from build123d import *

# Parameters (mm, degrees)
BASE_FLANGE_SKETCH_R = 11
BASE_FLANGE_DEPTH    = 24
HUB_BOSS_SKETCH_72_R = 36
HUB_BOSS_72_DEPTH    = 38
WEDGE_SUPPORT_DEPTH  = 28
BORE_28_REACH        = 176.416
BORE_SKETCH_28_R     = 14


with BuildPart() as part:
    # Base Flange Sketch → Base Flange (new body)
    with BuildSketch(Plane(origin=(0, 0, 0), x_dir=(1, 0, 0), z_dir=(0, 1, 0))):
        with BuildLine():
            Line((-116, 54.332778116), (-60, 54.332778116))
            ThreePointArc((-60, 54.332778116), (-42.391267518, 43.899782505), (-29.502831874, 28))
            Line((-29.502831874, 28), (0, 28))
            ThreePointArc((0, 28), (28, 0), (0, -28))
            Line((0, -28), (-29.502831874, -28))
            ThreePointArc((-29.502831874, -28), (-42.391267518, -43.899782505), (-60, -54.332778116))
            Line((-60, -54.332778116), (-116, -54.332778116))
            ThreePointArc((-116, -54.332778116), (-153.703467729, 0), (-116, 54.332778116))
        make_face()
        with Locations(Location((0, 0, 0), (0, 0, 270))):
            Circle(BASE_FLANGE_SKETCH_R, mode=Mode.SUBTRACT)
    extrude(amount=BASE_FLANGE_DEPTH)

    # Hub Boss Sketch Ø72 → Hub Boss Ø72 (add)
    with BuildSketch(Plane(origin=(0, 24, 0), x_dir=(1, 0, 0), z_dir=(0, 1, 0))):
        with Locations(Location((-88, 0, 0), (0, 0, 270))):
            Circle(HUB_BOSS_SKETCH_72_R)
    extrude(amount=HUB_BOSS_72_DEPTH)

    # Wedge Support Sketch → Wedge Support (add, symmetric)
    with BuildSketch(Plane(origin=(-88, 0, 0), x_dir=(0, 0, -1), z_dir=(1, 0, 0))):
        Polygon((-54.332778116, 24), (-13.504322415, 58.25914212), (13.266446181, 58.45874398), (54.332778116, 24), align=None)
    extrude(amount=WEDGE_SUPPORT_DEPTH, both=True)

    # Bore Sketch Ø28 → Bore Ø28 (cut, up to next)
    with BuildSketch(Plane(origin=(0, 62, 0), x_dir=(1, 0, 0), z_dir=(0, 1, 0)), mode=Mode.PRIVATE) as bore_28_sk1:
        with Locations(Location((-88, 0, 0), (0, 0, 270))):
            Circle(BORE_SKETCH_28_R)
    bore_28_tool1 = extrude(bore_28_sk1.sketch, amount=-BORE_28_REACH, mode=Mode.PRIVATE) & part.part
    add(bore_28_tool1.solids().sort_by_distance((-88, 62, 0))[0], mode=Mode.SUBTRACT)


solid = part.part
Source: CAD feature listing. Evaluate the final solid. Frame: model axes, mm. A direction names the side the tool comes from. Round coordinates to 2 decimals unless told otherwise and drop trailing zeros. Write each loop counter-clockwise with the first axis right and the second up, starting at its lowest first coordinate (ties: lowest second). Pieces come first, ordered by that corner, then holes. Notation, with made-up numbers: M 62.25,80.25 L 74.25,80.25 A32 ccw 74.25,111.25 Z; hole C 3.5,44 d5. An arc over 180 degrees is marked long. One line per item, written item: value. Start each with the question number.
Item 1: Ray query, L1, parallel to X at y = 8, z = 0; L2, parallel to Y at x = -53.5, z = -42; L3, parallel to Z at x = -99.5, y = 55. Return the intervals inside material, ascending. Write a range as from..to.
Item 2: Section query B-B (y = 13). Return the cut outline in (x, z).
Item 3: Section query D-D (z = -18). Return the cut outline in (x, y), plus the area to 3 significant figures.
Item 4: Section query C-C (x = -77). Return the cut outline in (y, z), plus the area to 3 significant figures.
Item 5: Set-up query: faces 1 (the flat face through (-15, 12, 28)), 2 (the cylindrical face through (-101.788, 46.956, 33.255)), 3 (the flat face through (-60, 32, -32)). Return all of +Z, -Z, +X, -X, +Y, -Y with unobstructed straight access to the full face (end or side cutting, diameter ignored); none if empty.
Item 6: Section query A-A (z = 0). Return the cut outline in (x, y), plus the area to 3 significant figures.
Item 7: Pin query (flat end, axial travel): pin 1 (8 mm diameter, centred on y = 35, z = -33.5, fed in from -X); pin 2 (19 mm diameter, centred on x = -11, y = 12.5, fed in from +Z); pin 3 (13.5 mm diameter, centred on y = 37.5, z = -43.5, fed in from +X). Return the tip coordinate at first contact, or that it passes through.
Item 8: Mould query, pull axis Z, two halves, no side actions, for faces 4 (the cylindrical face through (-74.12, 31.43, -1.82)), 5 (the cylindrical face through (-153.695, 11.832, 0.985)), 6 (the flat face through (-60, 32, 31)). Classes: pulls with the +Z half, pulls with the -Z half, needs draft (parallel to the pull), parting line crosses it, or undercut.
Result set:
1. L1: x = -153.7..-102, -74..-11, 11..28
1. L2: y = 0..24
1. L3: z = -34.11..-7.98, 7.98..34.11
2. outline: M -116,-54.33 L -60,-54.33 A58 ccw -29.5,-28 L 0,-28 A28 ccw 0,28 L -29.5,28 A58 ccw -60,54.33 L -116,54.33 A58 ccw Z; hole C -88,0 d28; hole C 0,0 d22
3. outline: M -150.84,0 L 21.45,0 L 21.45,24 L -56.82,24 L -56.82,62 L -119.18,62 L -119.18,24 L -150.84,24 Z
3. area: 6,500 mm²
4. outline: M 0,-54.33 L 24,-54.33 L 40.83,-34.28 L 62,-34.28 L 62,-8.66 L 0,-8.66 Z; M 0,8.66 L 62,8.66 L 62,34.28 L 40.83,34.28 L 24,54.33 L 0,54.33 Z
4. area: 4,480 mm²
5. face 1: +Z, +X, +Y, -Y
5. face 2: +Y
5. face 3: -Z, +X, +Y
6. outline: M -153.7,0 L -102,0 L -102,62 L -124,62 L -124,24 L -153.7,24 Z; M -74,0 L -11,0 L -11,24 L -52,24 L -52,62 L -74,62 Z; M 11,0 L 28,0 L 28,24 L 11,24 Z
6. area: 4,830 mm²
7. pin 1: stops at x = -116
7. pin 2: stops at z = 28
7. pin 3: stops at x = -60
8. face 4: undercut
8. face 5: parting line crosses it
8. face 6: needs draft
